Model file for the job. Use its own axes, mm. Coordinates: 2 decimals unless noted, no trailing zeros. Order: outer loops, then holes, each group sorted by start corner. A loop starts at its lowest first (then second) coordinate and runs counter-clockwise, first axis right, second up.
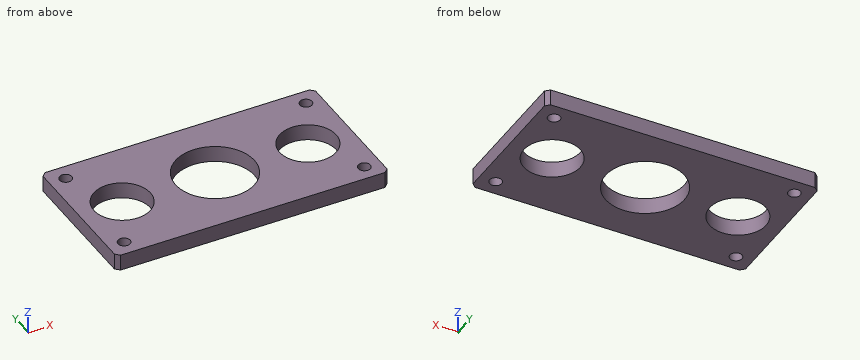
from build123d import *

# Parameters (mm, degrees)
SKETCH_1_W          = 135
SKETCH_1_H          = 70
EXTRUDE_1_DEPTH     = 8
CUT_EXTRUDE_1_REACH = 78.454
SKETCH_2_R          = 19.5
CUT_EXTRUDE_2_REACH = 78.454
SKETCH_3_R          = 14
CUT_EXTRUDE_3_REACH = 78.454
SKETCH_4_R          = 3
CHAMFER_1_SIZE      = 2


with BuildPart() as part:
    # 草图1 → 凸台-拉伸1 (new body)
    with BuildSketch(Plane.XY):
        Rectangle(SKETCH_1_W, SKETCH_1_H)
    extrude(amount=EXTRUDE_1_DEPTH)

    # 草图2 → 切除-拉伸1 (cut, up to next)
    with BuildSketch(Plane.XY.offset(8), mode=Mode.PRIVATE) as cut_extrude_1_sk1:
        Circle(SKETCH_2_R)
    cut_extrude_1_tool1 = extrude(cut_extrude_1_sk1.sketch, amount=-CUT_EXTRUDE_1_REACH, mode=Mode.PRIVATE) & part.part
    add(cut_extrude_1_tool1.solids().sort_by_distance((0, 0, 8))[0], mode=Mode.SUBTRACT)

    # 草图3 → 切除-拉伸2 (cut, up to next)
    with BuildSketch(Plane.XY.offset(8), mode=Mode.PRIVATE) as cut_extrude_2_sk1:
        with Locations((46, 0)):
            Circle(SKETCH_3_R)
    cut_extrude_2_tool1 = extrude(cut_extrude_2_sk1.sketch, amount=-CUT_EXTRUDE_2_REACH, mode=Mode.PRIVATE) & part.part
    # 草图3 → 切除-拉伸2 (cut, up to next)
    with BuildSketch(Plane.XY.offset(8), mode=Mode.PRIVATE) as cut_extrude_2_sk2:
        with Locations((-46, 0)):
            Circle(SKETCH_3_R)
    cut_extrude_2_tool2 = extrude(cut_extrude_2_sk2.sketch, amount=-CUT_EXTRUDE_2_REACH, mode=Mode.PRIVATE) & part.part
    add(cut_extrude_2_tool1.solids().sort_by_distance((46, 0, 8))[0], mode=Mode.SUBTRACT)
    add(cut_extrude_2_tool2.solids().sort_by_distance((-46, 0, 8))[0], mode=Mode.SUBTRACT)

    # 草图4 → 切除-拉伸3 (cut, up to next)
    with BuildSketch(Plane.XY.offset(8), mode=Mode.PRIVATE) as cut_extrude_3_sk1:
        with Locations((-59.5, 27)):
            Circle(SKETCH_4_R)
    cut_extrude_3_tool1 = extrude(cut_extrude_3_sk1.sketch, amount=-CUT_EXTRUDE_3_REACH, mode=Mode.PRIVATE) & part.part
    # 草图4 → 切除-拉伸3 (cut, up to next)
    with BuildSketch(Plane.XY.offset(8), mode=Mode.PRIVATE) as cut_extrude_3_sk2:
        with Locations((-59.5, -27)):
            Circle(SKETCH_4_R)
    cut_extrude_3_tool2 = extrude(cut_extrude_3_sk2.sketch, amount=-CUT_EXTRUDE_3_REACH, mode=Mode.PRIVATE) & part.part
    # 草图4 → 切除-拉伸3 (cut, up to next)
    with BuildSketch(Plane.XY.offset(8), mode=Mode.PRIVATE) as cut_extrude_3_sk3:
        with Locations(Location((59.5, -27, 0), (0, 0, 180))):
            Circle(SKETCH_4_R)
    cut_extrude_3_tool3 = extrude(cut_extrude_3_sk3.sketch, amount=-CUT_EXTRUDE_3_REACH, mode=Mode.PRIVATE) & part.part
    # 草图4 → 切除-拉伸3 (cut, up to next)
    with BuildSketch(Plane.XY.offset(8), mode=Mode.PRIVATE) as cut_extrude_3_sk4:
        with Locations(Location((59.5, 27, 0), (0, 0, 180))):
            Circle(SKETCH_4_R)
    cut_extrude_3_tool4 = extrude(cut_extrude_3_sk4.sketch, amount=-CUT_EXTRUDE_3_REACH, mode=Mode.PRIVATE) & part.part
    add(cut_extrude_3_tool1.solids().sort_by_distance((-59.5, 27, 8))[0], mode=Mode.SUBTRACT)
    add(cut_extrude_3_tool2.solids().sort_by_distance((-59.5, -27, 8))[0], mode=Mode.SUBTRACT)
    add(cut_extrude_3_tool3.solids().sort_by_distance((59.5, -27, 8))[0], mode=Mode.SUBTRACT)
    add(cut_extrude_3_tool4.solids().sort_by_distance((59.5, 27, 8))[0], mode=Mode.SUBTRACT)

    # 倒角1
    chamfer_1_edges = [part.edges().sort_by_distance(p)[0] for p in [
        (67.5, -35, 4),
        (-67.5, -35, 4),
        (-67.5, 35, 4),
        (67.5, 35, 4),
    ]]
    chamfer(chamfer_1_edges, length=CHAMFER_1_SIZE)


solid = part.part
Q1. Cut at B-B, the plane z = 2. List the corners of the cut face in (x, y), plus the area to 3 significant figures.
Established:
outline: (-67.5, -33) - (-65.5, -35) - (65.5, -35) - (67.5, -33) - (67.5, 33) - (65.5, 35) - (-65.5, 35) - (-67.5, 33) - close; hole circle Ø6 at (-59.5, -27); hole circle Ø6 at (-59.5, 27); hole circle Ø28 at (-46, 0); hole circle Ø39 at (0, 0); hole circle Ø28 at (46, 0); hole circle Ø6 at (59.5, -27); hole circle Ø6 at (59.5, 27)
area: 6,900 mm2
Q2. Cut at A-A, the plane y = 0. List the corners of the cut face in (x, z).
Established:
outline: (-67.5, 0) - (-60, 0) - (-60, 8) - (-67.5, 8) - close; (-32, 0) - (-19.5, 0) - (-19.5, 8) - (-32, 8) - close; (19.5, 0) - (32, 0) - (32, 8) - (19.5, 8) - close; (60, 0) - (67.5, 0) - (67.5, 8) - (60, 8) - close
Q3. Probe line 1 (X direction, y = 2, z = 5.25); line 2 (Y direction, x = -46, z = 5.75); line 3 (X direction, y = -11.5, z = 5). List the from-to ranges inside material, lowest first.
Established:
line 1: x = -67.5 to -59.86, -32.14 to -19.4, 19.4 to 32.14, 59.86 to 67.5
line 2: y = -35 to -14, 14 to 35
line 3: x = -67.5 to -53.98, -38.02 to -15.75, 15.75 to 38.02, 53.98 to 67.5
Q4. Cut at D-D, the plane x = 0. List the corners of the cut face in (y, z).
Established:
outline: (-35, 0) - (-19.5, 0) - (-19.5, 8) - (-35, 8) - close; (19.5, 0) - (35, 0) - (35, 8) - (19.5, 8) - close
Q5. Cut at C-C, the plane y = -27. List the corners of the cut face in (x, z).
Established:
outline: (-67.5, 0) - (-62.5, 0) - (-62.5, 8) - (-67.5, 8) - close; (-56.5, 0) - (56.5, 0) - (56.5, 8) - (-56.5, 8) - close; (62.5, 0) - (67.5, 0) - (67.5, 8) - (62.5, 8) - close
